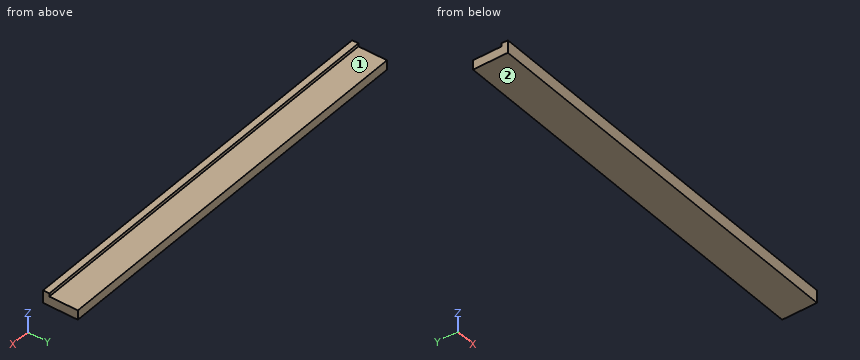
```python
from build123d import *

# Parameters (mm, degrees)
BOSS_EXTRUDE1_DEPTH = 630


with BuildPart() as part:
    # Sketch1 → Boss-Extrude1 (new body)
    with BuildSketch(Plane(origin=(0, 0, 0), x_dir=(0, 0, -1), z_dir=(1, 0, 0))):
        Polygon((-31.215474357, 48.108563949), (-31.215474357, -6.891436051), (-51.215474357, -6.891436051), (-51.215474357, 3.108563949), (-46.215474357, 3.108563949), (-46.215474357, 48.108563949), align=None)
    extrude(amount=-BOSS_EXTRUDE1_DEPTH)


solid = part.part
```
Input: part model. Units: mm. Frame: model coordinates. Face numbers are marked on the shaded views. A direction names the side the tool comes from. Round coordinates to 2 decimals unless told otherwise and drop trailing zeros. Write each loop counter-clockwise with the first axis right and the second up, starting at its lowest first coordinate (ties: lowest second). Pieces come first, ordered by that corner, then holes. Notation, with made-up numbers: (-6.75, 68) - (48.25, 68) arc R34 cw to (48.25, 106) - close; hole circle Ø7 at (88, -15.75). An arc over 180 degrees is marked (long way). Write item = value, one per line.
(1) Contact query for a flat-ended pin moving along its axis: pin 1 Ø4 at (x, z) = (-264.5, 48.5) entering from +Y. Output: stop coordinate, or through.
Geometry check:
pin_1 = 3.11
(2) Access query for the marked faces 1 and 2. Directions: +Z, -Z, +X, -X, +Y, -Y. A direction counts if a zero-diameter tool reaches every point of the face in a straight line with its end or side. Return the directions, or none.
Geometry check:
face_1 = +Z, +X, -X, +Y
face_2 = -Z, +X, -X, +Y, -Y
(3) Material intervals for probe 1 along Z at (x, y) = (-114, 24.5); probe 2 along Y at (x, z) = (-96, 49.5), sorted ascending.
Geometry check:
probe_1 = 31.22 to 46.22
probe_2 = -6.89 to 3.11
(4) Section query A-A on y = 25.5. Output: boundary loops of the cut face in (x, z), then the cut area to 3 significant figures.
Geometry check:
outline = (-630, 31.22) - (0, 31.22) - (0, 46.22) - (-630, 46.22) - close
area = 9,450 mm^2
(5) Section query B-B on x = -78. Output: boundary loops of the cut face in (y, z), then the cut area to 3 significant figures.
Geometry check:
outline = (-6.89, 31.22) - (48.11, 31.22) - (48.11, 46.22) - (3.11, 46.22) - (3.11, 51.22) - (-6.89, 51.22) - close
area = 875 mm^2
